Check sheet for the drawn part. Datum: minimum x, y, z corner. Units: mm. A direction names the side the tool comes from. Give positions to 0.01 mm unless a question says otherwise; leave off trailing zeros. Loops run counter-clockwise (first coordinate to the right, second up) from the corner with the lowest first, then second, coordinate; pieces in that order, holes last. Notation, with made-up numbers: (-40, 23) - (-13, 23) arc R23 cw to (-13, 42) - close; hole circle Ø9 at (31, 66). An arc over 180 degrees is marked (long way). Answer in a Markdown table with one row per item.
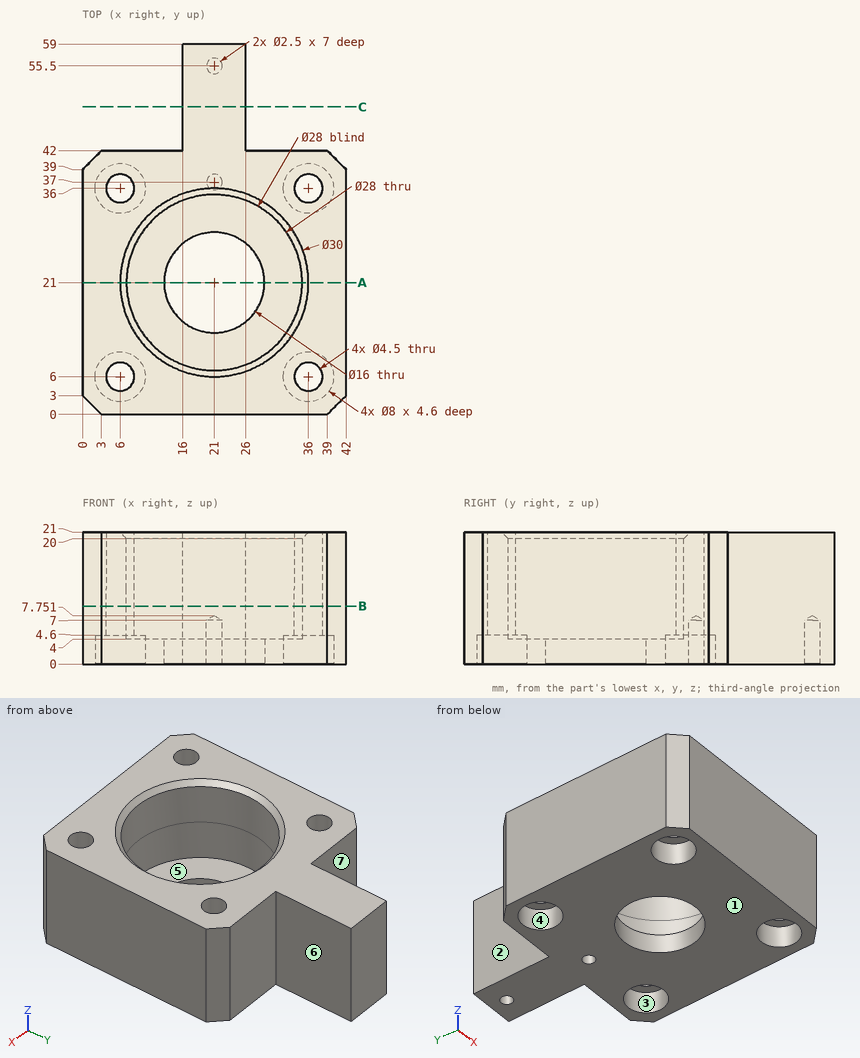
Q1. Go/stop test with flat-tipped pins: P1, Ø10.5, axis at x = 6.5, z = 8, coming from the +Y side; P2, Ø6.5, axis at x = 6, y = 36, coming from the -Z side; P3, Ø4, axis at x = 6, y = 6, coming from the -Z side; P4, Ø17, axis at x = 21, y = 21, coming from the +Z side. Record where each tip stops, or that it passes through.
Completed:
| item | result |
|---|---|
| P1 | y = 42 |
| P2 | z = 4.6 |
| P3 | through |
| P4 | z = 4 |
Q2. Sectioned sample at A-A (y = 21). Record the cut outline in (x, z), and give its area (3 significant figures).
Completed:
| item | result |
|---|---|
| outline | (0, 0) - (13, 0) - (13, 4) - (7, 4) - (7, 20) - (6, 21) - (0, 21) - close; (29, 0) - (42, 0) - (42, 21) - (36, 21) - (35, 20) - (35, 4) - (29, 4) - close |
| area | 341 mm^2 |
Q3. Draft check along X on the marked faces 1, 2 and 3. Enter one of: +X half, -X half, draft (parallel to the pull), parting line (faces both ways), or undercut.
Completed:
| item | result |
|---|---|
| face 1 | draft |
| face 2 | -X half |
| face 3 | undercut |
Q4. Sectioned sample at C-C (y = 49). Record the cut outline in (x, z), and give its area (3 significant figures).
Completed:
| item | result |
|---|---|
| outline | (16, 0) - (26, 0) - (26, 21) - (16, 21) - close |
| area | 210 mm^2 |
Q5. Thickness scan on line 1 (Y direction, x = 6, z = 1.1); line 2 (X direction, y = 36, z = 14.5); line 3 (X direction, y = 7, z = 2.5). Record the ranges inside material, lowest first.
Completed:
| item | result |
|---|---|
| line 1 | 0 to 2, 10 to 32, 40 to 42 |
| line 2 | 0 to 3.75, 8.25 to 33.75, 38.25 to 42 |
| line 3 | 0 to 2.13, 9.87 to 32.13, 39.87 to 42 |
Q6. Tool access check on the marked faces 4, 5, 6 and 7. Record the directions out of +Z, -Z, +X, -X, +Y, -Y that give a thin tool (end or side, any length) a straight path to the whole face; none if there is none.
Completed:
| item | result |
|---|---|
| face 4 | -Z |
| face 5 | +Z |
| face 6 | +Z, -Z, +X, +Y |
| face 7 | +Z, -Z, -X, +Y |
Q7. Sectioned sample at B-B (z = 9.25). Record the cut outline in (x, y), and give its area (3 significant figures).
Completed:
| item | result |
|---|---|
| outline | (0, 3) - (3, 0) - (39, 0) - (42, 3) - (42, 39) - (39, 42) - (26, 42) - (26, 59) - (16, 59) - (16, 42) - (3, 42) - (0, 39) - close; hole circle Ø4.5 at (6, 6); hole circle Ø4.5 at (6, 36); hole circle Ø28 at (21, 21); hole circle Ø4.5 at (36, 6); hole circle Ø4.5 at (36, 36) |
| area | 1,240 mm^2 |
